```python
from build123d import *

# Parameters (mm, degrees)
SKETCH1_R           = 75
BOSS_EXTRUDE1_DEPTH = 40
SKETCH2_R           = 8
CUT_EXTRUDE1_DEPTH  = 150
SKETCH10_R          = 100
CUT_EXTRUDE5_DEPTH  = 20
SKETCH11_R          = 30
SKETCH11_R_2        = 8
BOSS_EXTRUDE2_DEPTH = 20
SKETCH12_R          = 130
CUT_EXTRUDE6_DEPTH  = 30
SKETCH13_W          = 4
SKETCH13_H          = 4
CUT_EXTRUDE7_DEPTH  = 500
SKETCH15_W          = 3.4
SKETCH15_H          = 65


with BuildPart() as part:
    # Sketch1 → Boss-Extrude1 (new, symmetric)
    with BuildSketch(Plane.XY):
        Circle(SKETCH1_R)
    extrude(amount=BOSS_EXTRUDE1_DEPTH, both=True)

    # Sketch2 → Cut-Extrude1 (cut)
    with BuildSketch(Plane.XY.offset(40)):
        Circle(SKETCH2_R)
    extrude(amount=-CUT_EXTRUDE1_DEPTH, mode=Mode.SUBTRACT)

    # Sketch4 → Cut-Revolve1 (revolve, cut)
    with BuildSketch(Plane(origin=(0, 0, 0), x_dir=(0, 0, -1), z_dir=(1, 0, 0)), mode=Mode.PRIVATE) as cut_revolve1_sk:
        Polygon((-40, 75), (-36.6, 75), (-33.604349764, 66.3), (-26.395650236, 66.3), (-23.4, 75), (-21.6, 75), (-18.604349764, 66.3), (-11.395650236, 66.3), (-8.4, 75), (-6.6, 75), (-3.604349764, 66.3), (3.604349764, 66.3), (6.6, 75), (10, 75), (10, 161.050459045), (-40, 161.050459045), align=None)
    revolve(cut_revolve1_sk.sketch.rotate(Axis((0, 0, 0), (0, 0, -1)), 90), axis=Axis((0, 0, 0), (0, 0, -1)), mode=Mode.SUBTRACT)

    # Sketch10 → Cut-Extrude5 (cut)
    with BuildSketch(Plane(origin=(0, 0, -40), x_dir=(-1, 0, 0), z_dir=(0, 0, -1))):
        Circle(SKETCH10_R)
    extrude(amount=-CUT_EXTRUDE5_DEPTH, mode=Mode.SUBTRACT)

    # Sketch11 → Boss-Extrude2 (add)
    with BuildSketch(Plane(origin=(0, 0, -20), x_dir=(-1, 0, 0), z_dir=(0, 0, -1))):
        Circle(SKETCH11_R)
        with Locations(Location((0, 0, 0), (0, 0, 180))):
            Circle(SKETCH11_R_2, mode=Mode.SUBTRACT)
    extrude(amount=BOSS_EXTRUDE2_DEPTH)

    # Sketch12 → Cut-Extrude6 (cut)
    with BuildSketch(Plane(origin=(0, 0, -40), x_dir=(-1, 0, 0), z_dir=(0, 0, -1))):
        Circle(SKETCH12_R)
    extrude(amount=-CUT_EXTRUDE6_DEPTH, mode=Mode.SUBTRACT)

    # Sketch13 → Cut-Extrude7 (cut)
    with BuildSketch(Plane(origin=(0, 0, -10), x_dir=(-1, 0, 0), z_dir=(0, 0, -1))):
        with Locations((0, 8)):
            Rectangle(SKETCH13_W, SKETCH13_H)
    extrude(amount=-CUT_EXTRUDE7_DEPTH, mode=Mode.SUBTRACT)

    # Sketch15 → M8 Tapped Hole1 (revolve, cut)
    with BuildSketch(Plane(origin=(0, 10, 15), x_dir=(0, 0, -1), z_dir=(1, 0, 0))):
        with Locations((1.7, 32.5)):
            Rectangle(SKETCH15_W, SKETCH15_H)
    revolve(axis=Axis((0, 3.65, 15), (0, 1, 0)), mode=Mode.SUBTRACT)


solid = part.part
```
CAD build for the part. Positions are in the model's coordinates, mm. A direction names the side the tool comes from. Round coordinates to 2 decimals unless told otherwise and drop trailing zeros. Order: outer loops, then holes, each group sorted by start corner. A loop starts at its lowest first (then second) coordinate and runs counter-clockwise, first axis right, second up.
Item 1: Pin check, flat tips, straight feed: pin 1 (13 mm diameter, centred on x = 0, y = 0, fed in from +Z); pin 2 (5 mm diameter, centred on y = -51.5, z = 1, fed in from +X); pin 3 (6 mm diameter, centred on x = -18, z = 30, fed in from -Y); pin 4 (0.7 mm diameter, centred on x = -3, z = 15, fed in from +Y). Stop position of each tip, or through.
Item 2: Saw through at D-D on z = 15. Write the cut outline in (x, y), then the cut area to 3 significant figures.
Item 3: Tool access for faces 1 (the face through (0, 10, 29)), 2 (the face through (2.069, 38.544, 17.698)), 3 (the face through (-52.95, 40.6, 18.75)): list every direction of +Z, -Z, +X, -X, +Y, -Y with a clear straight run to the whole face (end or side of a thin tool).
Item 4: Probe line 1 along Y through (x, z) = (0, 23); line 2 along Z through (x, y) = (0, 37); line 3 along Z through (x, y) = (47, 47.5). List the from-to ranges inside material, lowest first.
Item 5: Mould opens along Z. For faces 4 (the face through (0, -8, 15)), 5 (the face through (-14.373, 64.723, 14.95)), 6 (the face through (16, 1, 40)), 7 (the face through (30.84, 59.3, 26.21)) say: pulls with the +Z half, pulls with the -Z half, needs draft (parallel to the pull), parting line crosses it, or undercut.
Item 6: Saw through at B-B on x = 0. State how many separate pieces and enclosed holes the cut face has, then the cut area to 3 significant figures.
Item 7: Saw through at C-C on z = -1. Write the cut outline in (x, y), then the cut area to 3 significant figures.
Reported:
1. pin 1: passes through
1. pin 2: stops at x = 44.66
1. pin 3: stops at y = -64.58
1. pin 4: stops at y = 10
2. outline: (-3.4, 10) - (-3.4, 66.21) arc R66.3 ccw (long way) to (3.4, 66.21) - (3.4, 10) - (2, 10) - (2, 7.75) arc R8 cw (long way) to (-2, 7.75) - (-2, 10) - close
2. area: 13,200 mm2
3. face 1: +Z, -Z
3. face 2: +Y
3. face 3: none
4. line 1: y = -75 to -8, 10 to 75
4. line 2: z = -10 to 11.6, 18.4 to 40
4. line 3: z = -10 to -3.78, 3.78 to 11.22, 18.78 to 26.22, 33.78 to 40
5. face 4: needs draft
5. face 5: undercut
5. face 6: pulls with the +Z half
5. face 7: undercut
6. separate pieces: 3
6. enclosed holes: 0
6. area: 5,680 mm2
7. outline: circle Ø132.6 at (0, 0); hole (-2, 7.75) arc R8 ccw (long way) to (2, 7.75) - (2, 10) - (-2, 10) - close
7. area: 13,600 mm2
